```python
from build123d import *

# Parameters (mm, degrees)
SKETCH_1_W               = 40
SKETCH_1_H               = 8
EXTRUDE_1_DEPTH          = 330.5
EXTRUDE_START            = -4
EXTRUDE_9_DEPTH          = 7.5
CUT_EXTRUDE_1_DEPTH      = 375.443041078
CUT_EXTRUDE_1_DEPTH_BACK = 375.443041078
SKETCH_14_R              = 17.5
EXTRUDE_10_DEPTH         = 40
SKETCH_16_W              = 176
SKETCH_16_H              = 3.5
EXTRUDE_11_DEPTH         = 40
SKETCH_17_W              = 176
SKETCH_17_H              = 3.5
EXTRUDE_12_DEPTH         = 40
FILLET_1_R               = 1
CUT_EXTRUDE_2_DEPTH      = 398.850950952
CUT_EXTRUDE_2_DEPTH_BACK = 398.850950952
EXTRUDE_13_DEPTH         = 40


with BuildPart() as part:
    # 草图1 → 凸台-拉伸1 (new, symmetric)
    with BuildSketch(Plane.XY):
        Rectangle(SKETCH_1_W, SKETCH_1_H)
    extrude(amount=EXTRUDE_1_DEPTH, both=True)

    # 草图13 → 凸台-拉伸9 (add, symmetric)
    with BuildSketch(Plane.XZ.offset(4).offset(EXTRUDE_START)):
        with BuildLine():
            Line((153.622249649, 33.30434644), (20, 88))
            Line((20, 88), (20, -88))
            Line((20, -88), (153.998078719, -31.322105093))
            ThreePointArc((153.998078719, -31.322105093), (175.362862221, 1.116458369), (153.622249649, 33.30434644))
        make_face()
    extrude(amount=EXTRUDE_9_DEPTH, both=True)

    # 草图14 → 切除-拉伸1 (cut, two sides: drawn at the far end of the back side and taken through both)
    with BuildSketch(Plane.XZ.offset(7.5).offset(-CUT_EXTRUDE_1_DEPTH_BACK)):
        with Locations(Location((140.363454038, 0.912922591, 0), (0, 0, 270))):
            Circle(SKETCH_14_R)
    extrude(amount=CUT_EXTRUDE_1_DEPTH + CUT_EXTRUDE_1_DEPTH_BACK, mode=Mode.SUBTRACT)

    # 草图15 → 凸台-拉伸10 (add)
    with BuildSketch(Plane.ZY.offset(20)):
        Polygon((330.5, 4), (333.5, 4), (333.5, 6), (343.5, 6), (343.5, 4), (346.5, 4), (346.5, 0.516928803), (346.5, -4), (343.5, -4), (343.5, -6), (333.5, -6), (333.5, -4), (330.5, -4), align=None)
    extrude_10 = extrude(amount=-EXTRUDE_10_DEPTH)

    # 草图16 → 凸台-拉伸11 (add)
    with BuildSketch(Plane.ZY.offset(-20)):
        with Locations((0, 5.75)):
            Rectangle(SKETCH_16_W, SKETCH_16_H)
    extrude(amount=EXTRUDE_11_DEPTH)

    # 草图17 → 凸台-拉伸12 (add)
    with BuildSketch(Plane.ZY.offset(-20)):
        with Locations((0, -5.75)):
            Rectangle(SKETCH_17_W, SKETCH_17_H)
    extrude(amount=EXTRUDE_12_DEPTH)

    # 镜向1: 凸台-拉伸10 across plane
    add(extrude_10.mirror(Plane.XY))

    # 圆角1
    fillet_1_edges = [part.edges().sort_by_distance(p)[0] for p in [
        (0, 4, 88),
        (0, 4, -88),
        (0, -4, -88),
        (0, -4, 88),
    ]]
    fillet(fillet_1_edges, radius=FILLET_1_R)

    # 草图18 → 切除-拉伸2 (cut, two sides: drawn at the far end of the back side and taken through both)
    with BuildSketch(Plane.ZY.offset(20).offset(-CUT_EXTRUDE_2_DEPTH_BACK)):
        Polygon((-339.5, 4), (-339.5, 6), (-343.5, 6), (-343.5, 4), (-346.5, 4), (-346.5, -4), (-343.5, -4), (-343.5, -6), (-339.5, -6), (-339.5, -4), (-342.5, -4), (-342.5, 4), align=None)
    extrude(amount=CUT_EXTRUDE_2_DEPTH + CUT_EXTRUDE_2_DEPTH_BACK, mode=Mode.SUBTRACT)

    # 草图19 → 凸台-拉伸13 (add)
    with BuildSketch(Plane.ZY.offset(20)):
        Polygon((-332.5, 4), (-332.5, 6), (-342.5, 6), (-342.5, -6), (-332.5, -6), (-332.5, -4), align=None)
    extrude(amount=-EXTRUDE_13_DEPTH)


solid = part.part
```
For this review, take the finished solid that the model builds, in its own axes (mm). A direction names the side the tool comes from. Round coordinates to 2 decimals unless told otherwise and drop trailing zeros. Write each loop counter-clockwise with the first axis right and the second up, starting at its lowest first coordinate (ties: lowest second). Pieces come first, ordered by that corner, then holes. Notation, with made-up numbers: M 50,53 L 85,53 A9 cw 85,67 Z; hole C 15.25,47.25 d7. An arc over 180 degrees is marked long. One line per item, written item: value. Start each with the question number.
(1) We need section B-B (y = 0). Give the boundary of the cut face in (x, z), and give its area (3 significant figures).
(2) The part is to be moulded in two halves that separate along Z. For faces 1 (the flat face through (0, -4, 213)), 2 (the flat face through (0, 4, -209)), 3 (the flat face through (-20, 0, -3)), 4 (the cylindrical face through (175.36, -0.11, 0.54)), say which applies: released by +Z, released by -Z, zero draft, split by the parting line, or undercut.
(3) Insertion check: pin 1 (5 mm diameter, centred on x = 132.5, y = -3, fed in from -Z); pin 2 (12 mm diameter, centred on x = 39, z = -86, fed in from -Y); pin 3 (3.5 mm diameter, centred on y = -1.5, z = -192.5, fed in from +X); pin 4 (8 mm diameter, centred on x = 22, z = 128, fed in from -Y). Each pin has a flat end and moves straight along its axis. Give the tip position at first contact, or say it passes through.
(4) We need section A-A (x = 2). Give the boundary of the cut face in (y, z).
(5) Wall thickness on line 1 (X direction, y = 3.75, z = 173.5); line 2 (Z direction, x = 148, y = -1.75); line 3 (Z direction, x = 147, y = -2.75): over which ranges is each line inside the solid? List them lowest first.
(6) Machinability: for faces 5 (the flat face through (0, -4, -212)), 6 (the flat face through (20, 0, -217)), 7 (the flat face through (20, 0, 219)), 8 (the flat face through (0, 4, 210)), which of the approach directions +Z, -Z, +X, -X, +Y, -Y give a long, thin tool a straight path to every point of the face, cutting with its end or side? Answer none if there is none.
(7) We need section D-D (x = 99). Give the boundary of the cut face in (y, z), and give its area (3 significant figures).
(8) We need section C-C (z = -105.5). Give the boundary of the cut face in (x, y), and give its area (3 significant figures).
Result:
1. outline: M -20,-342.5 L 20,-342.5 L 20,-88 L 154,-31.32 A35 ccw 153.62,33.3 L 20,88 L 20,346.5 L -20,346.5 Z; hole C 140.36,0.91 d35
1. area: 43,700 mm²
2. face 1: undercut
2. face 2: undercut
2. face 3: zero draft
2. face 4: split by the parting line
3. pin 1: z = -41.47
3. pin 2: y = -7.5
3. pin 3: x = 20
3. pin 4: y = -4
4. outline: M -7.5,-88 L -5,-88 A1 cw -4,-89 L -4,-332.5 L -6,-332.5 L -6,-342.5 L 6,-342.5 L 6,-332.5 L 4,-332.5 L 4,-89 A1 cw 5,-88 L 7.5,-88 L 7.5,88 L 5,88 A1 cw 4,89 L 4,333.5 L 6,333.5 L 6,343.5 L 4,343.5 L 4,346.5 L -4,346.5 L -4,343.5 L -6,343.5 L -6,333.5 L -4,333.5 L -4,89 A1 cw -5,88 L -7.5,88 Z
5. line 1: -20 to 20
5. line 2: -33.86 to -14.83, 16.66 to 35.61
5. line 3: -34.28 to -15.28, 17.11 to 36.02
6. face 5: +X, -X, -Y
6. face 6: -Z, +X, +Y, -Y
6. face 7: +Z, +X, +Y, -Y
6. face 8: +X, -X, +Y
7. outline: M -7.5,-54.58 L 7.5,-54.58 L 7.5,55.66 L -7.5,55.66 Z
7. area: 1,650 mm²
8. outline: M -20,-4 L 20,-4 L 20,4 L -20,4 Z
8. area: 320 mm²
